Could you check a few things on this drawing? It's one solid part, dimensions in mm from its lowest x, y, z. A direction names the side the tool comes from. Coordinates: 2 decimals unless noted, no trailing zeros. Loops run counter-clockwise (first coordinate to the right, second up) from the corner with the lowest first, then second, coordinate; pieces in that order, holes last. Notation, with made-up numbers: M 25,86 L 61,86 A23 ccw 61,113 Z; hole C 77.25,-0.5 d4. An arc over 180 degrees is marked long. Use one line per item in the form item = value. Start each with the question number.
(1) Imagine slicing it at D-D, the plane z = 30. Please give me the cut outline in (x, y).
(2) Thinking about a two-plate mould opening in X: for the marked faces 3, 4 and 5, which applies, +X half, -X half, draft (parallel to the pull), parting line (faces both ways), or undercut?
(3) Will these pins go through, and if not, where does the flat tip stop? P1, Ø4, axis at x = 20, y = 12, coming from the +Z side; P2, Ø8.5, axis at x = 5, y = 12, coming from the -Z side; P3, Ø12.5, axis at x = 11.5, z = 15.5, coming from the -Y side.
(4) Imagine slicing it at C-C, the plane x = 12.5. Please give me the cut outline in (y, z).
(5) Please list where these lines run through material, in increasing order: L1, parallel to X at y = 37, z = 10; L2, parallel to Y at x = 5, z = 35.5; L3, parallel to Z at x = 12.5, y = 39.
(6) On a 3-axis mill with a long thin cutter (end or side, diameter ignored), from which of +Z, -Z, +X, -X, +Y, -Y can I reach the whole of each face in a straight line? I mean the marked faces 1 and 2. Say none if no direction works.
(7) Imagine slicing it at B-B, the plane z = 10. Please give me the cut outline in (x, y).
(8) Imagine slicing it at A-A, the plane y = 12. Please give me the cut outline in (x, z).
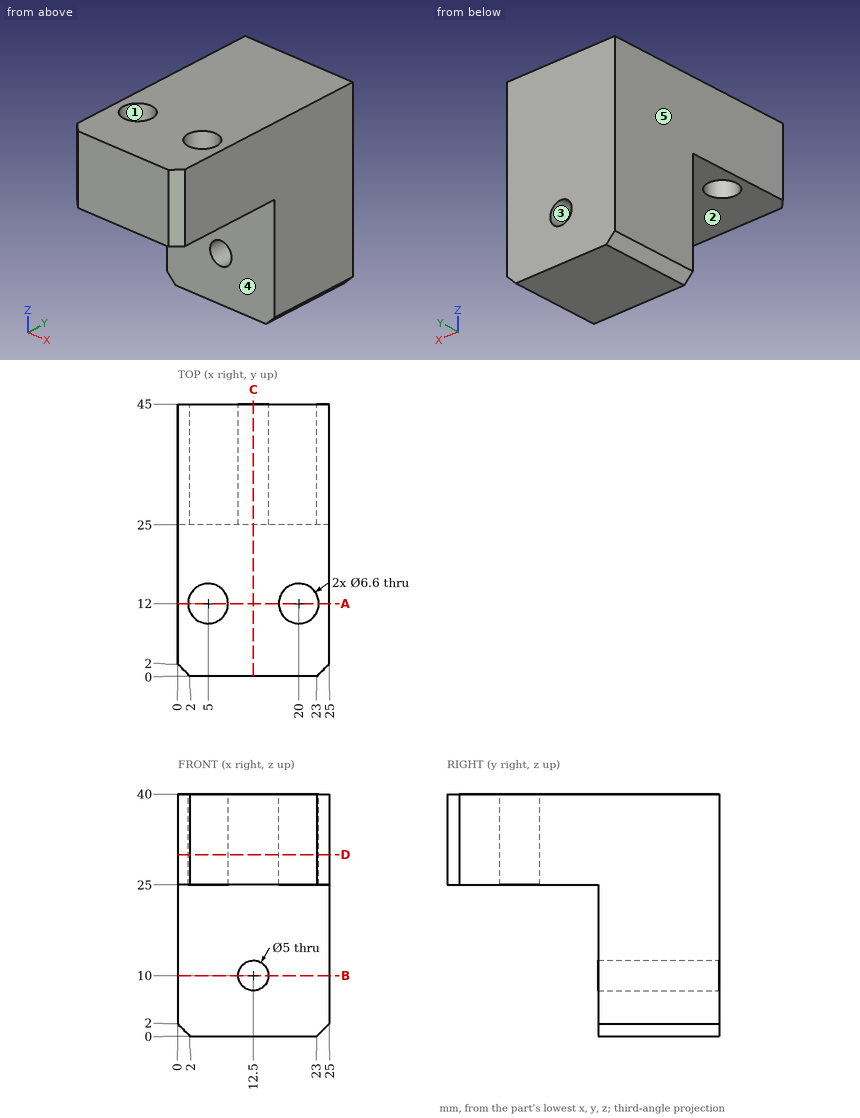
Answer:
q1.outline = M 0,2 L 2,0 L 23,0 L 25,2 L 25,45 L 0,45 Z; hole C 5,12 d6.6; hole C 20,12 d6.6
q2.face_3 = undercut
q2.face_4 = draft
q2.face_5 = -X half
q3.P1 = through
q3.P2 = 25
q3.P3 = 25
q4.outline = M 0,25 L 25,25 L 25,12.5 L 45,12.5 L 45,40 L 0,40 Z; M 25,0 L 45,0 L 45,7.5 L 25,7.5 Z
q5.L1 = 0 to 10, 15 to 25
q5.L2 = 0 to 8.7, 15.3 to 45
q5.L3 = 0 to 7.5, 12.5 to 40
q6.face_1 = +Z, -Z
q6.face_2 = -Z, +X, -X, -Y
q7.outline = M 0,25 L 10,25 L 10,45 L 0,45 Z; M 15,25 L 25,25 L 25,45 L 15,45 Z
q8.outline = M 0,25 L 1.7,25 L 1.7,40 L 0,40 Z; M 8.3,25 L 16.7,25 L 16.7,40 L 8.3,40 Z; M 23.3,25 L 25,25 L 25,40 L 23.3,40 Z
